```python
from build123d import *

# Parameters (mm, degrees)
EXTRUDE_1_DEPTH        = 63
FILLET_1_R             = 10
FILLET_2_R             = 1.5
SKETCH_2_R             = 1.5
CUT_EXTRUDE_1_DEPTH    = 10
SKETCH_3_W             = 11.5
SKETCH_3_H             = 31
EXTRUDE_2_DEPTH        = 6.5
FILLET_3_R             = 4
HOLE_WIZARD_M3_1_D     = 2.5
HOLE_WIZARD_M3_1_DEPTH = 11.5
HOLE_WIZARD_M3_1_TIP   = 0.751075774
SKETCH_6_W             = 45
SKETCH_6_H             = 70
SKETCH_6_H_2           = 75
CUT_EXTRUDE_2_DEPTH    = 10


with BuildPart() as part:
    # 草图1 → 凸台-拉伸1 (new, symmetric)
    with BuildSketch(Plane.XY):
        Polygon((0, 140), (0, 0), (202.5, 0), (202.5, 67), (126, 67), (126, 140), align=None)
    extrude(amount=EXTRUDE_1_DEPTH, both=True)

    # 圆角1
    fillet_1_edges = [part.edges().sort_by_distance(p)[0] for p in [
        (126, 140, 0),
        (0, 140, 0),
    ]]
    fillet(fillet_1_edges, radius=FILLET_1_R)

    # 圆角2
    fillet_2_edges = [part.edges().sort_by_distance(p)[0] for p in [
        (202.5, 67, 0),
    ]]
    fillet(fillet_2_edges, radius=FILLET_2_R)

    # 草图2 → 切除-拉伸1 (cut)
    with BuildSketch(Plane(origin=(0, 67, 0), x_dir=(1, 0, 0), z_dir=(0, 1, 0))):
        with Locations(Location((194.22, 0.5, 0), (0, 0, 180))):
            Circle(SKETCH_2_R)
    extrude(amount=-CUT_EXTRUDE_1_DEPTH, mode=Mode.SUBTRACT)

    # 草图3 → 凸台-拉伸2 (add)
    with BuildSketch(Plane(origin=(0, 67, 0), x_dir=(1, 0, 0), z_dir=(0, 1, 0))):
        with Locations((195.75, -38)):
            Rectangle(SKETCH_3_W, SKETCH_3_H)
        with Locations((195.75, 31)):
            Rectangle(SKETCH_3_W, SKETCH_3_H)
    extrude(amount=EXTRUDE_2_DEPTH)

    # 圆角3
    fillet_3_edges = [part.edges().sort_by_distance(p)[0] for p in [
        (126, 67, 0),
    ]]
    fillet(fillet_3_edges, radius=FILLET_3_R)

    # M3 螺纹孔1
    with Locations(Plane(origin=(0, 0, 0), x_dir=(-1, 0, 0), z_dir=(0, -1, 0))):
        with Locations((-16, -35), (-16, 35), (-186.5, -45), (-186.5, 45)):
            Hole(HOLE_WIZARD_M3_1_D / 2, depth=HOLE_WIZARD_M3_1_DEPTH)
            with Locations((0, 0, -(HOLE_WIZARD_M3_1_DEPTH + HOLE_WIZARD_M3_1_TIP / 2))):  # 118° drill point
                Cone(0, HOLE_WIZARD_M3_1_D / 2, HOLE_WIZARD_M3_1_TIP, mode=Mode.SUBTRACT)

    # 草图6 → 切除-拉伸2 (cut)
    with BuildSketch(Plane(origin=(0, 0, 0), x_dir=(-1, 0, 0), z_dir=(0, -1, 0))):
        with Locations((-76.5, 10)):
            Rectangle(SKETCH_6_W, SKETCH_6_H)
        with Locations((-142, -6.5)):
            Rectangle(SKETCH_6_W, SKETCH_6_H_2)
    extrude(amount=-CUT_EXTRUDE_2_DEPTH, mode=Mode.SUBTRACT)


solid = part.part
```
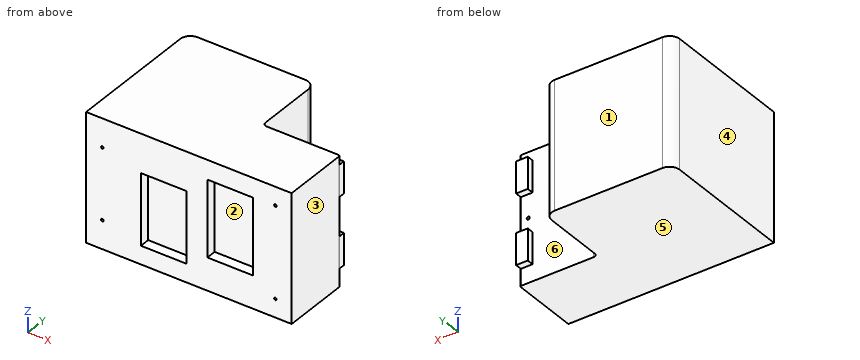
The model under review builds one solid part; all positions refer to its coordinate system, in mm. Face numbers are marked on the shaded views. A direction names the side the tool comes from. Coordinates: 2 decimals unless noted, no trailing zeros. Loops run counter-clockwise (first coordinate to the right, second up) from the corner with the lowest first, then second, coordinate; pieces in that order, holes last. Notation, with made-up numbers: (-20.75, 88.5) -> (22.25, 88.5) arc R15 cw to (22.25, 100.5) -> close; hole circle Ø7 at (-12, 16.25). An arc over 180 degrees is marked (long way). Answer as CSV lines item,"result".
Item 1: Insertion check: pin 1 (5 mm diameter, centred on y = 72, z = -29, fed in from +X); pin 2 (13.5 mm diameter, centred on x = 71, z = 1.5, fed in from -Y); pin 3 (12 mm diameter, centred on y = 92.5, z = -16, fed in from +X). Each pin has a flat end and moves straight along its axis. Give the tip position at first contact, or say it passes through.
Results below:
pin 1,"stops at x = 201.5"
pin 2,"stops at y = 10"
pin 3,"stops at x = 126"
Item 2: Take a section at C-C, the plane y = 98. State the section outline as (x, z) points, and give its area (3 significant figures).
Results below:
outline,"(0, -63) -> (126, -63) -> (126, 63) -> (0, 63) -> close"
area,"15,900 mm2"
Item 3: Machinability: for the marked faces 1 and 2, which of the approach directions +Z, -Z, +X, -X, +Y, -Y give a long, thin tool a straight path to every point of the face, cutting with its end or side? Answer none if there is none.
Results below:
face 1,"+Z, -Z, +X, -X, +Y"
face 2,"-Y"
Item 4: For L1, parallel to Z at x = 16, y = 4.5; L2, parallel to X at y = 9, z = 35; L3, parallel to X at y = 4, z = -35, list the stretches that pass through material, from the lowest coordinate up.
Results below:
L1,"z = -63 to -36.25, -33.75 to 33.75, 36.25 to 63"
L2,"x = 0 to 14.75, 17.25 to 119.5, 164.5 to 202.5"
L3,"x = 0 to 14.75, 17.25 to 54, 99 to 202.5"
Item 5: Draft analysis for pull direction X (two halves, no side actions). For the marked faces 3, 4, 5 and 6, state which applies: +X half, -X half, draft (parallel to the pull), parting line (faces both ways), or undercut.
Results below:
face 3,"+X half"
face 4,"-X half"
face 5,"draft"
face 6,"undercut"
Item 6: Take a section at D-D, the plane x = 58. State the section outline as (y, z) points.
Results below:
outline,"(0, -63) -> (140, -63) -> (140, 63) -> (0, 63) -> (0, 25) -> (10, 25) -> (10, -45) -> (0, -45) -> close"
Item 7: Take a section at A-A, the plane x = 139.5. State the section outline as (y, z) points.
Results below:
outline,"(0, -63) -> (67, -63) -> (67, 63) -> (0, 63) -> (0, 44) -> (10, 44) -> (10, -31) -> (0, -31) -> close"
Item 8: Take a section at B-B, the plane z = -25.5. State the section outline as (x, y) points, and give its area (3 significant figures).
Results below:
outline,"(0, 0) -> (54, 0) -> (54, 10) -> (99, 10) -> (99, 0) -> (119.5, 0) -> (119.5, 10) -> (164.5, 10) -> (164.5, 0) -> (202.5, 0) -> (202.5, 65.5) arc R1.5 ccw to (201, 67) -> (201.5, 67) -> (201.5, 73.5) -> (190, 73.5) -> (190, 67) -> (130, 67) arc R4 cw to (126, 71) -> (126, 130) arc R10 ccw to (116, 140) -> (10, 140) arc R10 ccw to (0, 130) -> close"
area,"21,900 mm2"
